```python
from build123d import *

# Parameters (mm, degrees)
BOSS_EXTRUDE1_DEPTH = 10
SKETCH2_W           = 14
SKETCH2_H           = 30
BOSS_EXTRUDE2_DEPTH = 30
BOSS_EXTRUDE4_DEPTH = 5
SKETCH5_W           = 6
SKETCH5_H           = 7
BOSS_EXTRUDE5_DEPTH = 6
SKETCH6_W           = 15
SKETCH6_H           = 15
BOSS_EXTRUDE6_DEPTH = 14
SKETCH7_R           = 1
CUT_EXTRUDE1_DEPTH  = 2
FILLET1_R           = 1
SKETCH8_R           = 1.5
SKETCH8_W           = 21.297654542
SKETCH8_H           = 29.54423259
CUT_EXTRUDE2_DEPTH  = 10
SKETCH9_W           = 4
SKETCH9_H           = 12
CUT_EXTRUDE3_DEPTH  = 7.5
SKETCH11_R          = 1.5
SKETCH11_W          = 46.682021109
SKETCH11_H          = 78.101327177
CUT_EXTRUDE6_DEPTH  = 50
SKETCH12_W          = 25.193851166
SKETCH12_H          = 16.960566472
CUT_EXTRUDE7_DEPTH  = 20
FILLET2_R           = 3
SKETCH13_W          = 3
SKETCH13_H          = 6
CUT_EXTRUDE8_DEPTH  = 20
SKETCH14_R          = 11.800022464
CUT_EXTRUDE9_DEPTH  = 3
SKETCH15_R          = 1.5
BOSS_EXTRUDE7_DEPTH = 1
SKETCH16_R          = 4.865347009
SKETCH16_R_2        = 1.5
CUT_EXTRUDE10_DEPTH = 2
FILLET5_R           = 1


with BuildPart() as part:
    # Sketch1 → Boss-Extrude1 (new body)
    with BuildSketch(Plane.XY):
        Polygon((0, 0), (15, 0), (9.79055467, 29.54423259), (20.05115897, 57.735011214), (10.05115897, 57.735011214), (2.497462604, 29.54423259), (8.920552671, 5.572934119), (0, 4), align=None)
    boss_extrude1 = extrude(amount=BOSS_EXTRUDE1_DEPTH)

    # Sketch2 → Boss-Extrude2 (add)
    with BuildSketch(Plane.XY.offset(10)):
        with Locations((15.05115897, 72.735011214)):
            Rectangle(SKETCH2_W, SKETCH2_H)
    extrude(amount=-BOSS_EXTRUDE2_DEPTH)

    # Sketch4 → Boss-Extrude4 (add)
    with BuildSketch(Plane.XY.offset(10)):
        Polygon((15.05115897, 84.235011214), (30.372047832, 71.37925902), (30.372047832, 56.37925902), (27.30787006, 56.37925902), (27.30787006, 68.950409459), (15.05115897, 79.235011214), align=None)
    boss_extrude4 = extrude(amount=BOSS_EXTRUDE4_DEPTH)

    # Mirror1: Boss-Extrude1, Boss-Extrude4 across plane
    add(boss_extrude1.mirror(Plane.XY.offset(-5)))
    add(boss_extrude4.mirror(Plane.XY.offset(-5)))

    # Sketch5 → Boss-Extrude5 (add)
    with BuildSketch(Plane(origin=(0, 87.735011214, 0), x_dir=(1, 0, 0), z_dir=(0, 1, 0))):
        with Locations((15.05115897, 5)):
            Rectangle(SKETCH5_W, SKETCH5_H)
    extrude(amount=BOSS_EXTRUDE5_DEPTH)

    # Sketch6 → Boss-Extrude6 (add)
    with BuildSketch(Plane(origin=(0, 93.735011214, 0), x_dir=(1, 0, 0), z_dir=(0, 1, 0))):
        with Locations((15.05115897, 5)):
            Rectangle(SKETCH6_W, SKETCH6_H)
    extrude(amount=BOSS_EXTRUDE6_DEPTH)

    # Sketch7 → Cut-Extrude1 (cut)
    with BuildSketch(Plane.ZY.offset(-7.55115897)):
        with Locations((-8.96, 103.735011214)):
            Circle(SKETCH7_R)
        with Locations(Location((-1.04, 103.735011214, 0), (0, 0, 180))):
            Circle(SKETCH7_R)
    extrude(amount=-CUT_EXTRUDE1_DEPTH, mode=Mode.SUBTRACT)

    # Fillet1
    fillet1_edges = [part.edges().sort_by_distance(p)[0] for p in [
        (18.55115897, 81.298162505, 10),
        (15.05115897, 81.735011214, 10),
        (15.05115897, 84.235011214, 12.5),
        (18.55115897, 76.298162505, 10),
        (15.05115897, 79.235011214, 12.5),
        (18.55115897, 81.298162505, -20),
        (18.55115897, 76.298162505, -20),
        (15.05115897, 81.735011214, -20),
        (15.05115897, 79.235011214, -22.5),
        (15.05115897, 84.235011214, -22.5),
    ]]
    fillet(fillet1_edges, radius=FILLET1_R)

    # Sketch8 → Cut-Extrude2 (cut)
    with BuildSketch(Plane(origin=(0, 0, -20), x_dir=(-1, 0, 0), z_dir=(0, 0, -1))):
        with Locations((-7.157843169, 32.54423259)):
            Circle(SKETCH8_R)
        with Locations((-4.351172729, 14.772116295)):
            Rectangle(SKETCH8_W, SKETCH8_H)
    extrude(amount=-CUT_EXTRUDE2_DEPTH, mode=Mode.SUBTRACT)

    # Sketch9 → Cut-Extrude3 (cut, symmetric)
    with BuildSketch(Plane.ZY.offset(-8.05115897)):
        with Locations((-15, 30.54423259)):
            Rectangle(SKETCH9_W, SKETCH9_H)
    extrude(amount=CUT_EXTRUDE3_DEPTH, both=True, mode=Mode.SUBTRACT)

    # Sketch11 → Cut-Extrude6 (cut, symmetric)
    with BuildSketch(Plane(origin=(0, 0, -20), x_dir=(-1, 0, 0), z_dir=(0, 0, -1))):
        with Locations(Location((-7.157843169, 32.54423259, 0), (0, 0, 180))):
            Circle(SKETCH11_R)
        with Locations((-27.446168312, 74.594896179)):
            Rectangle(SKETCH11_W, SKETCH11_H)
    extrude(amount=CUT_EXTRUDE6_DEPTH, both=True, mode=Mode.SUBTRACT)


with BuildPart() as cut_extrude6_piece_1:
    # of the separate pieces the step leaves, piece 1, a body of its own (cut_extrude6_pieces)
    add(part.part.solids().sort_by_distance((4.105157758, 35.54423259, 10))[0])

    # Fillet2
    fillet2_edges = [cut_extrude6_piece_1.edges().sort_by_distance(p)[0] for p in [
        (11.974376076, 35.54423259, 5),
        (4.105157758, 35.54423259, 5),
    ]]
    fillet(fillet2_edges, radius=FILLET2_R)

    # Sketch13 → Cut-Extrude8 (cut)
    with BuildSketch(Plane(origin=(0, 0, 0), x_dir=(0, 0, -1), z_dir=(1, 0, 0))):
        with Locations((-8.5, 32.54423259)):
            Rectangle(SKETCH13_W, SKETCH13_H)
        with Locations((-1.5, 32.54423259)):
            Rectangle(SKETCH13_W, SKETCH13_H)
    extrude(amount=CUT_EXTRUDE8_DEPTH, mode=Mode.SUBTRACT)

    # Sketch14 → Cut-Extrude9 (cut)
    with BuildSketch(Plane(origin=(0, 0, 0), x_dir=(-1, 0, 0), z_dir=(0, 0, -1))):
        with Locations((-6.144008637, 37.54423259)):
            Circle(SKETCH14_R)
    cut_extrude9 = extrude(amount=-CUT_EXTRUDE9_DEPTH, mode=Mode.SUBTRACT)

    # Mirror2: Cut-Extrude9 across plane
    add(cut_extrude9.mirror(Plane(origin=(0, 0, 5), x_dir=(1, 0, 0), z_dir=(0, 0, -1))), mode=Mode.SUBTRACT)

    # Sketch15 → Boss-Extrude7 (add)
    with BuildSketch(Plane.XY.offset(10)):
        with Locations((11.303234902, 3.163151803)):
            Circle(SKETCH15_R)
    extrude(amount=BOSS_EXTRUDE7_DEPTH)

    # Sketch16 → Cut-Extrude10 (cut)
    with BuildSketch(Plane.XY.offset(10)):
        with Locations((11.303234902, 3.163151803)):
            Circle(SKETCH16_R)
        with Locations((11.303234902, 3.163151803)):
            Circle(SKETCH16_R_2, mode=Mode.SUBTRACT)
    extrude(amount=-CUT_EXTRUDE10_DEPTH, mode=Mode.SUBTRACT)

    # Fillet5
    fillet5_edges = [cut_extrude6_piece_1.edges().sort_by_distance(p)[0] for p in [
        (6.891812395, 5.215212471, 9),
        (13.695196152, 7.399910339, 9),
        (8.500606317, 7.140195245, 9),
        (7.606469803, 0, 9),
    ]]
    fillet(fillet5_edges, radius=FILLET5_R)


with BuildPart() as cut_extrude6_piece_2:
    # of the separate pieces the step leaves, piece 2, a body of its own (cut_extrude6_pieces)
    add(part.part.solids().sort_by_distance((4.105157758, 35.54423259, -20))[0])


with BuildPart() as cut_extrude6_piece_3:
    # of the separate pieces the step leaves, piece 3, a body of its own (cut_extrude6_pieces)
    add(part.part.solids().sort_by_distance((4.105157758, 35.54423259, -10))[0])


with BuildPart() as cut_extrude7_tool:
    # Sketch12 → Cut-Extrude7 (new body)
    with BuildSketch(Plane(origin=(0, 0, -20), x_dir=(-1, 0, 0), z_dir=(0, 0, -1))):
        with Locations((-9.102890418, 33.861350945)):
            Rectangle(SKETCH12_W, SKETCH12_H)
    extrude(amount=-CUT_EXTRUDE7_DEPTH)


with BuildPart() as cut_extrude6_piece_2_1:
    add(cut_extrude6_piece_2.part)

    # Cut-Extrude7: cut by cut_extrude7_tool
    add(cut_extrude7_tool.part, mode=Mode.SUBTRACT)


with BuildPart() as cut_extrude6_piece_3_1:
    add(cut_extrude6_piece_3.part)

    # Cut-Extrude7: cut by cut_extrude7_tool
    add(cut_extrude7_tool.part, mode=Mode.SUBTRACT)


solid = cut_extrude6_piece_1.part
```
The model under review builds one solid part; all positions refer to its coordinate system, in mm. A direction names the side the tool comes from. Coordinates: 2 decimals unless noted, no trailing zeros. Write each loop counter-clockwise with the first axis right and the second up, starting at its lowest first coordinate (ties: lowest second). Pieces come first, ordered by that corner, then holes. Notation, with made-up numbers: (8, -34) - (62, -34) arc R24 ccw to (62, -22) - close; hole circle Ø9 at (58.25, 33). An arc over 180 degrees is marked (long way). Answer in a Markdown table with one row per item. Add a question column.
Q1. Consider section D-D on z = 3.5. Give the boundary of the cut face in (x, y).
Q2. For faces 4 (the face through (6.961, 25.773, 8.521)), 5 (the face through (8.681, 7.727, 9.014)), 6 (the face through (3, 3, 10)), list the 3-axis set-ups (+Z, -Z, +X, -X, +Y, -Y) from which the entire face can be reached by the end or side of a thin tool; tool diameter is ignored.
Q3. To check wall thickness, follow line 1 along Z through (x, y) = (6.25, 1.5); line 2 along Z through (x, y) = (8.75, 29); line 3 along Y through (x, z) = (2.5, 2.75). State the ranges of each line that lie inside material, in increasing order. Write a range as from..to.
Q4. Consider section C-C on x = 11.5. Give the boundary of the cut face in (y, z), then the cut area to 3 significant figures.
Q5. Draft analysis for pull direction X (two halves, no side actions). For faces 1 (the face through (8.589, 32.094, 4.972)), 2 (the face through (10.145, 30.517, 4.972)), 3 (the face through (8, 17, 10)), state which applies: +X half, -X half, draft (parallel to the pull), parting line (faces both ways), or undercut.
Q6. Consider section B-B on z = 8.5. Give the boundary of the cut face in (x, y), then the cut area to 3 significant figures.
Q7. Consider section A-A on x = 4.25. Give the boundary of the cut face in (y, z).
Q8. Clearance check with flat-ended pins moving along their axes: pin 1 (2.5 mm diameter, centred on x = 7, y = 28.5, fed in from +Z); pin 2 (1.5 mm diameter, centred on x = 2.5, y = 2, fed in from +Z); pin 3 (5 mm diameter, centred on x = 11.5, z = 3, fed in from +Y); pin 4 (1 mm diameter, centred on y = 28.5, z = 2, fed in from -X). State where each tip first meets the part, or that it passes through.
Answers below:
| question | item | result |
|---|---|---|
| 1 | outline | (0, 0) - (15, 0) - (9.79, 29.54) - (10.51, 31.52) arc R3 ccw to (7.69, 35.54) - (6.41, 35.54) arc R3 ccw to (3.51, 33.32) - (2.5, 29.54) - (8.92, 5.57) - (0, 4) - close; hole circle Ø3 at (7.16, 32.54) |
| 2 | face 4 | +Z, +Y |
| 2 | face 5 | +Z, -Y |
| 2 | face 6 | +Z, -X, +Y, -Y |
| 3 | line 1 | 0..10 |
| 3 | line 2 | 3..7 |
| 3 | line 3 | 0..4.44 |
| 4 | outline | (0, 0) - (19.85, 0) - (19.85, 10) - (8.02, 10) - (8.02, 8) - (4.65, 8) - (4.65, 11) - (1.68, 11) - (1.68, 8) - (0, 8) - close |
| 4 | area | 191 mm² |
| 5 | face 1 | undercut |
| 5 | face 2 | +X half |
| 5 | face 3 | draft |
| 6 | outline | (0, 0) - (5.85, 0) arc R1 ccw to (6.78, 1.37) arc R4.87 cw to (6.48, 3.82) arc R1 ccw to (5.32, 4.94) - (0, 4) - close; (3.43, 26.06) - (8.17, 8.36) arc R1 ccw to (9.51, 7.69) arc R4.87 cw to (12.22, 7.94) arc R1 ccw to (13.4, 9.1) - (10.33, 26.51) arc R11.8 cw to start; circle Ø3 at (11.3, 3.16) |
| 6 | area | 147 mm² |
| 7 | outline | (0, 0) - (4.75, 0) - (4.75, 10) - (0, 10) - close; (23, 0) - (25.9, 0) - (25.9, 3) - (34.63, 3) - (34.63, 7) - (25.9, 7) - (25.9, 10) - (23, 10) - close |
| 8 | pin 1 | z = 7 |
| 8 | pin 2 | z = 10 |
| 8 | pin 3 | y = 35.24 |
| 8 | pin 4 | through |
